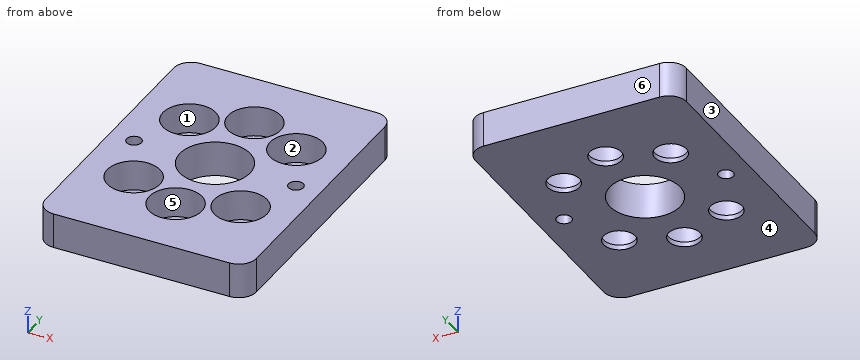
```python
from build123d import *

# Parameters (mm, degrees)
SKETCH1_W                                           = 60
SKETCH1_H                                           = 80
SKETCH1_R                                           = 10
SKETCH1_R_2                                         = 2
BOSS_EXTRUDE1_DEPTH                                 = 10
M5_TAPPED_HOLE1_D                                   = 4.2
CBORE_FOR_M8_HEX_SOCKET_HEAD_CAP_SCREW1_D           = 9
CBORE_FOR_M8_HEX_SOCKET_HEAD_CAP_SCREW1_CBORE_D     = 15
CBORE_FOR_M8_HEX_SOCKET_HEAD_CAP_SCREW1_CBORE_DEPTH = 8.6
CIRPATTERN1_COUNT                                   = 8
FILLET1_R                                           = 5


with BuildPart() as part:
    # Sketch1 → Boss-Extrude1 (new body)
    with BuildSketch(Plane.XY):
        Rectangle(SKETCH1_W, SKETCH1_H)
        Circle(SKETCH1_R, mode=Mode.SUBTRACT)
        with Locations((-23, 0)):
            Circle(SKETCH1_R_2, mode=Mode.SUBTRACT)
        with Locations(Location((23, 0, 0), (0, 0, 180))):
            Circle(SKETCH1_R_2, mode=Mode.SUBTRACT)
    extrude(amount=BOSS_EXTRUDE1_DEPTH)

    # M5 Tapped Hole1 (through all)
    with Locations(Plane.XY.offset(10)):
        with Locations((-23, 0), (23, 0)):
            Hole(M5_TAPPED_HOLE1_D / 2)

    # CBORE for M8 Hex Socket Head Cap Screw1 (through all)
    with Locations(Plane.XY.offset(10)):
        with Locations((0, 21.5)):
            cbore_for_m8_hex_socket_head_cap_screw1 = CounterBoreHole(CBORE_FOR_M8_HEX_SOCKET_HEAD_CAP_SCREW1_D / 2, CBORE_FOR_M8_HEX_SOCKET_HEAD_CAP_SCREW1_CBORE_D / 2, CBORE_FOR_M8_HEX_SOCKET_HEAD_CAP_SCREW1_CBORE_DEPTH)

    # CirPattern1: CBORE for M8 Hex Socket Head Cap Screw1 ×8 about axis, 2 skipped
    cirpattern1_axis = Axis((0, 0, 0), (0, 0, 1))
    add([cbore_for_m8_hex_socket_head_cap_screw1.rotate(cirpattern1_axis, i * 360 / CIRPATTERN1_COUNT) for i in range(1, CIRPATTERN1_COUNT) if i not in (2, 6)], mode=Mode.SUBTRACT)

    # Fillet1
    fillet1_edges = [part.edges().sort_by_distance(p)[0] for p in [
        (30, -40, 5),
        (-30, -40, 5),
        (-30, 40, 5),
        (30, 40, 5),
    ]]
    fillet(fillet1_edges, radius=FILLET1_R)


solid = part.part
```
The model under review builds one solid part; all positions refer to its coordinate system, in mm. Face numbers are marked on the shaded views. A direction names the side the tool comes from. Give positions to 0.01 mm unless a question says otherwise; leave off trailing zeros. Write each loop counter-clockwise with the first axis right and the second up, starting at its lowest first coordinate (ties: lowest second). Pieces come first, ordered by that corner, then holes. Notation, with made-up numbers: M 49.25,-34 L 53.25,-34 A21 cw 53.25,-24 Z; hole C 44.25,-22 d10. An arc over 180 degrees is marked long. Answer in a Markdown table with one row per item.
Item 1: Add section A-A on y = 0. Give the boundary of the cut face in (x, z), plus the area to 3 significant figures.
Check sheet entries:
| item | result |
|---|---|
| outline | M -30,0 L -25.1,0 L -25.1,10 L -30,10 Z; M -20.9,0 L -10,0 L -10,10 L -20.9,10 Z; M 10,0 L 20.9,0 L 20.9,10 L 10,10 Z; M 25.1,0 L 30,0 L 30,10 L 25.1,10 Z |
| area | 316 mm2 |
Item 2: Tool access review of the marked faces 5 and 6: name each direction out of +Z, -Z, +X, -X, +Y, -Y from which nothing blocks a thin tool from reaching the whole face with its end or side.
Check sheet entries:
| item | result |
|---|---|
| face 5 | +Z |
| face 6 | +Z, -Z, +X, -X, +Y |
Item 3: For line 1 along Y through (x, z) = (0, 8); line 2 along Y through (x, z) = (0, 0.7); line 3 along X through (y, z) = (15.5, 1), list the stretches that pass through material, from the lowest coordinate up.
Check sheet entries:
| item | result |
|---|---|
| line 1 | -40 to -29, -14 to -10, 10 to 14, 29 to 40 |
| line 2 | -40 to -26, -17 to -10, 10 to 17, 26 to 40 |
| line 3 | -30 to -19.69, -10.71 to 10.71, 19.69 to 30 |
Item 4: Add section C-C on y = 21.5. Give the boundary of the cut face in (x, z).
Check sheet entries:
| item | result |
|---|---|
| outline | M -30,0 L -4.5,0 L -4.5,1.4 L -7.5,1.4 L -7.5,10 L -11.13,10 L -11.13,1.4 L -19.28,1.4 L -19.28,10 L -30,10 Z; M 4.5,0 L 30,0 L 30,10 L 19.28,10 L 19.28,1.4 L 11.13,1.4 L 11.13,10 L 7.5,10 L 7.5,1.4 L 4.5,1.4 Z |
Item 5: Add section B-B on x = 0. Give the boundary of the cut face in (y, z), plus the area to 3 significant figures.
Check sheet entries:
| item | result |
|---|---|
| outline | M -40,0 L -26,0 L -26,1.4 L -29,1.4 L -29,10 L -40,10 Z; M -17,0 L -10,0 L -10,10 L -14,10 L -14,1.4 L -17,1.4 Z; M 10,0 L 17,0 L 17,1.4 L 14,1.4 L 14,10 L 10,10 Z; M 26,0 L 40,0 L 40,10 L 29,10 L 29,1.4 L 26,1.4 Z |
| area | 317 mm2 |
Item 6: For P1, Ø5.5, axis at x = 15.2, y = 15.2, coming from the +Z side; P2, Ø7.5, axis at x = -12.5, y = 16.5, coming from the +Z side, all flat-tipped, find the tip position at first contact; note any pin that passes through.
Check sheet entries:
| item | result |
|---|---|
| P1 | through |
| P2 | z = 1.4 |
Item 7: Draft analysis for pull direction X (two halves, no side actions). For the marked faces 1, 2, 3 and 4, state which applies: +X half, -X half, draft (parallel to the pull), parting line (faces both ways), or undercut.
Check sheet entries:
| item | result |
|---|---|
| face 1 | undercut |
| face 2 | undercut |
| face 3 | -X half |
| face 4 | draft |
Item 8: Add section D-D on x = -16. Give the boundary of the cut face in (y, z), plus the area to 3 significant figures.
Check sheet entries:
| item | result |
|---|---|
| outline | M -40,0 L -19.63,0 L -19.63,1.4 L -22.66,1.4 L -22.66,10 L -40,10 Z; M -10.77,0 L 10.77,0 L 10.77,1.4 L 7.75,1.4 L 7.75,10 L -7.75,10 L -7.75,1.4 L -10.77,1.4 Z; M 19.63,0 L 40,0 L 40,10 L 22.66,10 L 22.66,1.4 L 19.63,1.4 Z |
| area | 519 mm2 |
